The listing builds one solid part. Answer for the finished solid, in the listing's coordinates (mm). A direction names the side the tool comes from. Coordinates: 2 decimals unless noted, no trailing zeros. Order: outer loops, then holes, each group sorted by start corner. A loop starts at its lowest first (then second) coordinate and runs counter-clockwise, first axis right, second up. Notation, with made-up numbers: (32.25, -31) - (42.25, -31) arc R15 cw to (42.25, -16) - close; hole circle Ø1 at (20, 45). An arc over 180 degrees is marked (long way). Use a Markdown table: item, result. Add a question column.
Item 1: For faces 4 (the cylindrical face through (0, 15, 55)), 5 (the flat face through (37, 0, -18)), 6 (the flat face through (-38, 3, 0)), 7 (the cylindrical face through (28.26, 32.47, 28.31)), determine the directions among +Z, -Z, +X, -X, +Y, -Y from which every point of the face is accessible in a straight line to the end or side of a thin tool.
Item 2: Flat-ended cylindrical pins translate along their axes: P1, Ø18, axis at y = 14, z = -73.5, coming from the +X side; P2, Ø1, axis at y = 12.5, z = 29.5, coming from the +X side; P3, Ø15.5, axis at x = -44.5, y = -4, coming from the -Z side. Find the tip coordinate at first contact, or state that the pin passes through.
Item 3: Find the intervals of material crossed by line 1 along Y through (x, z) = (-36, 20.5); line 2 along X through (y, z) = (-8.5, 6); line 3 along X through (y, z) = (-19.5, 16), in increasing order.
Item 4: The part is cut by section A-A, the plane x = 0. Give the vertices of the cut face in (y, z).
Item 5: The part is cut by section C-C, the plane x = -22.5. Give the vertices of the cut face in (y, z).
Item 6: The part is cut by section D-D, the plane x = 60. Give the vertices of the cut face in (y, z).
Item 7: The part is cut by section B-B, the plane z = -68. Give the vertices of the cut face in (x, y).
Item 8: The mould has two halves that part along Z. Classify faces 1 (the cylindrical face through (69.315, 15.21, 4.845)), 2 (the cylindrical face through (82.865, 15.21, 2.486)), 3 (the cylindrical face through (-59.8, 15.2, 10.5)): released by +Z, released by -Z, zero draft, split by the parting line, or undercut.
from build123d import *

# Parameters (mm, degrees)
HUB_TUBE_SKETCH_R        = 40
HUB_TUBE_SKETCH_R_2      = 30
HUB_TUBE_80_DEPTH        = 30
FLANGE_30MM_DEPTH        = 30
COLLAR_SKETCH_R          = 40
COLLAR_SKETCH_R_2        = 30
COLLAR_80_X5_DEPTH       = 5
SIDE_SLOT_CUT_DEPTH      = 135
SIDE_SLOT_CUT_DEPTH_BACK = 140
CUT_21_A_DEPTH           = 99
CUT_21_A_DEPTH_BACK      = 159
CUT_21_A_SKETCH_R        = 10.5
CUT_21_B_DEPTH           = 507
CUT_21_B_DEPTH_BACK      = 405
CUT_21_B_SKETCH_R        = 10.5


with BuildPart() as part:
    # Hub Tube Sketch → Hub Tube Ø80 (new, symmetric)
    with BuildSketch(Plane(origin=(0, 0, 0), x_dir=(1, 0, 0), z_dir=(0, 1, 0))):
        with Locations(Location((0, 0, 0), (0, 0, 270))):
            Circle(HUB_TUBE_SKETCH_R)
        with Locations(Location((0, 0, 0), (0, 0, 270))):
            Circle(HUB_TUBE_SKETCH_R_2, mode=Mode.SUBTRACT)
    extrude(amount=HUB_TUBE_80_DEPTH, both=True)

    # Flange Profile Sketch → Flange 30mm (add)
    with BuildSketch(Plane(origin=(0, 30, 0), x_dir=(1, 0, 0), z_dir=(0, 1, 0))):
        with BuildLine():
            ThreePointArc((-75.738459529, 16.772027059), (-82.895108188, -2.194087755), (-72.266666667, -19.455818895))
            Line((-72.266666667, -19.455818895), (-29.333333333, -46.524784315))
            ThreePointArc((-29.333333333, -46.524784315), (0, -55), (29.333333333, -46.524784315))
            Line((29.333333333, -46.524784315), (72.266666667, -19.455818895))
            ThreePointArc((72.266666667, -19.455818895), (82.895108188, -2.194087755), (75.738459529, 16.772027059))
            Line((75.738459529, 16.772027059), (41.314383018, 49.074737583))
            ThreePointArc((41.314383018, 49.074737583), (36.646358132, 55.712799721), (35, 63.659108939))
            Line((35, 63.659108939), (35, 80))
            Line((35, 80), (-35, 80))
            Line((-35, 80), (-35, 63.659108939))
            ThreePointArc((-35, 63.659108939), (-36.646358132, 55.712799721), (-41.314383018, 49.074737583))
            Line((-41.314383018, 49.074737583), (-75.738459529, 16.772027059))
        make_face()
        with BuildLine():
            ThreePointArc((40, 0), (-28.284271247, -28.284271247), (0, 40))
            ThreePointArc((0, 40), (28.284271247, 28.284271247), (40, 0))
        make_face(mode=Mode.SUBTRACT)
    extrude(amount=-FLANGE_30MM_DEPTH)

    # Collar Sketch → Collar Ø80 x5 (add)
    with BuildSketch(Plane(origin=(0, 30, 0), x_dir=(1, 0, 0), z_dir=(0, 1, 0))):
        with Locations(Location((0, 0, 0), (0, 0, 270))):
            Circle(COLLAR_SKETCH_R)
        with Locations(Location((0, 0, 0), (0, 0, 270))):
            Circle(COLLAR_SKETCH_R_2, mode=Mode.SUBTRACT)
    extrude(amount=COLLAR_80_X5_DEPTH)

    # Side Slot Sketch → Side Slot Cut (cut, two sides: drawn at the far end of the back side and taken through both)
    with BuildSketch(Plane.XZ.offset(-SIDE_SLOT_CUT_DEPTH_BACK)):
        Polygon((-109.161413969, 0), (-2.593057922, 0), (-2.593057922, -87.129471891), (-109.161413969, -88.900340716), align=None)
    extrude(amount=SIDE_SLOT_CUT_DEPTH + SIDE_SLOT_CUT_DEPTH_BACK, mode=Mode.SUBTRACT)

    # Cut Ø21 A Sketch → Cut Ø21 A (cut, two sides: drawn at the far end of the back side and taken through both)
    with BuildSketch(Plane.XZ.offset(-CUT_21_A_DEPTH_BACK)):
        with Locations(Location((60, 0, 0), (0, 0, 90))):
            Circle(CUT_21_A_SKETCH_R)
    extrude(amount=CUT_21_A_DEPTH + CUT_21_A_DEPTH_BACK, mode=Mode.SUBTRACT)

    # Cut Ø21 B Sketch → Cut Ø21 B (cut, two sides: drawn at the far end of the back side and taken through both)
    with BuildSketch(Plane.XZ.offset(-CUT_21_B_DEPTH_BACK)):
        with Locations((-60, 0)):
            Circle(CUT_21_B_SKETCH_R)
    extrude(amount=CUT_21_B_DEPTH + CUT_21_B_DEPTH_BACK, mode=Mode.SUBTRACT)


solid = part.part
Solution:
| question | item | result |
|---|---|---|
| 1 | face 4 | +Z, +Y, -Y |
| 1 | face 5 | -Y |
| 1 | face 6 | -Z, -X, +Y, -Y |
| 1 | face 7 | +Y |
| 2 | P1 | stops at x = 35 |
| 2 | P2 | stops at x = 57.13 |
| 2 | P3 | stops at z = 0 |
| 3 | line 1 | y = 0 to 30 |
| 3 | line 2 | x = -39.55 to -29.39, 29.39 to 39.55 |
| 3 | line 3 | x = -36.66 to -25.38, 25.38 to 36.66 |
| 4 | outline | (-30, -40) - (0, -40) - (0, -80) - (30, -80) - (30, -40) - (35, -40) - (35, -30) - (-30, -30) - close; (-30, 30) - (35, 30) - (35, 40) - (30, 40) - (30, 55) - (0, 55) - (0, 40) - (-30, 40) - close |
| 5 | outline | (-30, 19.84) - (35, 19.84) - (35, 33.07) - (30, 33.07) - (30, 50.19) - (0, 50.19) - (0, 33.07) - (-30, 33.07) - close |
| 6 | outline | (0, -31.54) - (30, -31.54) - (30, -10.5) - (0, -10.5) - close; (0, 10.5) - (30, 10.5) - (30, 27.19) - (0, 27.19) - close |
| 7 | outline | (-2.59, 0) - (35, 0) - (35, 30) - (-2.59, 30) - close |
| 8 | face 1 | undercut |
| 8 | face 2 | split by the parting line |
| 8 | face 3 | released by -Z |
